The model under review builds one solid part; all positions refer to its coordinate system, in mm. A direction names the side the tool comes from. Round coordinates to 2 decimals unless told otherwise and drop trailing zeros. Order: outer loops, then holes, each group sorted by start corner. A loop starts at its lowest first (then second) coordinate and runs counter-clockwise, first axis right, second up.
```python
from build123d import *

# Parameters (mm, degrees)
BASE_BLOCK_80X80X40_DEPTH = 40
COUNTERBORE_1_SKETCH_R    = 20
COUNTERBORE_1_40X10_DEPTH = 10
BORE_1_SKETCH_R           = 10
BORE_1_20_DEPTH           = 30
SIDE_BOSS_DEPTH           = 30
SIDE_BOSS_TRIM_CUT_DEPTH  = 30
COUNTERBORE_2_SKETCH_R    = 20
COUNTERBORE_2_40X10_DEPTH = 10
BORE_2_SKETCH_R           = 10
BORE_2_20_DEPTH           = 30
GUSSET_1_DEPTH            = 10
GUSSET_2_DEPTH            = 10


with BuildPart() as part:
    # Base Block Sketch → Base Block 80x80x40 (new body)
    with BuildSketch(Plane.XY):
        with BuildLine():
            Line((0, 40), (60, 40))
            ThreePointArc((60, 40), (100, 0), (60, -40))
            Line((60, -40), (0, -40))
            ThreePointArc((0, -40), (-40, 0), (0, 40))
        make_face()
    extrude(amount=BASE_BLOCK_80X80X40_DEPTH)

    # Counterbore 1 Sketch → Counterbore 1 Ø40x10 (cut)
    with BuildSketch(Plane.XY.offset(40)):
        Circle(COUNTERBORE_1_SKETCH_R)
    extrude(amount=-COUNTERBORE_1_40X10_DEPTH, mode=Mode.SUBTRACT)

    # Bore 1 Sketch → Bore 1 Ø20 (cut)
    with BuildSketch(Plane.XY.offset(30)):
        Circle(BORE_1_SKETCH_R)
    extrude(amount=-BORE_1_20_DEPTH, mode=Mode.SUBTRACT)

    # Side Boss Sketch → Side Boss (add)
    with BuildSketch(Plane.XY.offset(40)):
        with BuildLine():
            Line((60, 40), (60, -40))
            ThreePointArc((60, -40), (100, 0), (60, 40))
        make_face()
    extrude(amount=SIDE_BOSS_DEPTH)

    # Side Boss Trim Sketch → Side Boss Trim Cut (cut)
    with BuildSketch(Plane.XY.offset(70)):
        with BuildLine():
            Line((60, 20), (60, -20))
            ThreePointArc((60, -20), (80, 0), (60, 20))
        make_face()
    extrude(amount=-SIDE_BOSS_TRIM_CUT_DEPTH, mode=Mode.SUBTRACT)

    # Counterbore 2 Sketch → Counterbore 2 Ø40x10 (cut)
    with BuildSketch(Plane.XY.offset(40)):
        with Locations((60, 0)):
            Circle(COUNTERBORE_2_SKETCH_R)
    extrude(amount=-COUNTERBORE_2_40X10_DEPTH, mode=Mode.SUBTRACT)

    # Bore 2 Sketch → Bore 2 Ø20 (cut)
    with BuildSketch(Plane.XY.offset(30)):
        with Locations((60, 0)):
            Circle(BORE_2_SKETCH_R)
    extrude(amount=-BORE_2_20_DEPTH, mode=Mode.SUBTRACT)

    # Gusset 1 Sketch → Gusset 1 (add)
    with BuildSketch(Plane.XZ.offset(40)):
        Polygon((60, 70), (60, 40), (30, 40), align=None)
    extrude(amount=-GUSSET_1_DEPTH)

    # Gusset 2 Sketch → Gusset 2 (add)
    with BuildSketch(Plane(origin=(0, 40, 0), x_dir=(1, 0, 0), z_dir=(0, 1, 0))):
        Polygon((60, -70), (60, -40), (30, -40), align=None)
    extrude(amount=-GUSSET_2_DEPTH)


solid = part.part
```
(1) For faces 1 (the flat face through (22, 1, 40)), 2 (the cylindrical face through (79.005, -6.23, 50.28)), 3 (the flat face through (31, 1, 0)), list the 3-axis set-ups (+Z, -Z, +X, -X, +Y, -Y) from which the entire face can be reached by the end or side of a thin tool; tool diameter is ignored.
Data:
face 1: +Z, -X
face 2: +Z
face 3: -Z, +X, -X, +Y, -Y
(2) Draft analysis for pull direction Y (two halves, no side actions). For faces 4 (the cylindrical face through (99.99, -0.88, 34.51)), 5 (the flat face through (60, 25, 55)), 6 (the flat face through (84, 1, 70)), state which applies: pulls with the +Y half, pulls with the -Y half, needs draft (parallel to the pull), parting line crosses it, or undercut.
Data:
face 4: parting line crosses it
face 5: undercut
face 6: needs draft
(3) Consider section A-A (y = 0). Write out the cut boundary in (x, z), and give its area (3 significant figures).
Data:
outline: (-40, 0) - (-10, 0) - (-10, 30) - (-20, 30) - (-20, 40) - (-40, 40) - close; (10, 0) - (50, 0) - (50, 30) - (40, 30) - (40, 40) - (20, 40) - (20, 30) - (10, 30) - close; (70, 0) - (100, 0) - (100, 70) - (80, 70) - (80, 30) - (70, 30) - close
area: 4,200 mm2
(4) Consider section B-B (z = 38). Write out the cut boundary in (x, y), and give its area (3 significant figures).
Data:
outline: (0, -40) - (60, -40) arc R40 ccw to (60, 40) - (0, 40) arc R40 ccw to start; hole circle Ø40 at (0, 0); hole circle Ø40 at (60, 0)
area: 7,310 mm2
(5) Insertion check: pin 1 (4 mm diameter, centred on x = 27, y = -28.5, fed in from -Z); pin 2 (2 mm diameter, centred on y = 13, z = 49.5, fed in from +X); pin 3 (3 mm diameter, centred on y = -25, z = 58.5, fed in from -X); pin 4 (5 mm diameter, centred on y = 16.5, z = 12, fed in from +X). Each pin has a flat end and moves straight along its axis. Give the tip position at first contact, or say it passes through.
Data:
pin 1: stops at z = 0
pin 2: stops at x = 98.16
pin 3: stops at x = 60
pin 4: stops at x = 97.47
(6) Consider section C-C (x = 55). Write out the cut boundary in (y, z), and give its area (3 significant figures).
Data:
outline: (-40, 0) - (-8.66, 0) - (-8.66, 30) - (-19.36, 30) - (-19.36, 40) - (-30, 40) - (-30, 65) - (-40, 65) - close; (8.66, 0) - (40, 0) - (40, 65) - (30, 65) - (30, 40) - (19.36, 40) - (19.36, 30) - (8.66, 30) - close
area: 2,790 mm2
(7) To check wall thickness, follow probe 1 along Y at (x, z) = (60, 15); probe 2 along X at (y, z) = (3, 11); probe 3 along X at (y, z) = (5.5, 15). State the ranges of each line that lie inside material, in increasing order.
Data:
probe 1: y = -40 to -10, 10 to 40
probe 2: x = -39.89 to -9.54, 9.54 to 50.46, 69.54 to 99.89
probe 3: x = -39.62 to -8.35, 8.35 to 51.65, 68.35 to 99.62
(8) Consider section D-D (z = 49.5). Write out the cut boundary in (x, y).
Data:
outline: (39.5, -40) - (60, -40) arc R40 ccw to (60, 40) - (39.5, 40) - (39.5, 30) - (60, 30) - (60, 20) arc R20 cw to (60, -20) - (60, -30) - (39.5, -30) - close
